from build123d import *

# Parameters (mm, degrees)
SKETCH_1_R             = 10
EXTRUDE_1_DEPTH        = 177
HOLE_WIZARD_M8_1_D     = 6.8
HOLE_WIZARD_M8_1_DEPTH = 19.75
HOLE_WIZARD_M8_1_TIP   = 2.042926105
HOLE_WIZARD_M8_2_D     = 6.8
HOLE_WIZARD_M8_2_DEPTH = 19.75
HOLE_WIZARD_M8_2_TIP   = 2.042926105
CHAMFER_1_SIZE         = 1


with BuildPart() as part:
    # 草图1 → 凸台-拉伸1 (new, symmetric)
    with BuildSketch(Plane.XY):
        Circle(SKETCH_1_R)
    extrude(amount=EXTRUDE_1_DEPTH, both=True)

    # M8 螺纹孔1
    with Locations(Plane(origin=(0, 0, -177), x_dir=(-1, 0, 0), z_dir=(0, 0, -1))):
        with Locations((0, 0)):
            Hole(HOLE_WIZARD_M8_1_D / 2, depth=HOLE_WIZARD_M8_1_DEPTH)
            with Locations((0, 0, -(HOLE_WIZARD_M8_1_DEPTH + HOLE_WIZARD_M8_1_TIP / 2))):  # 118° drill point
                Cone(0, HOLE_WIZARD_M8_1_D / 2, HOLE_WIZARD_M8_1_TIP, mode=Mode.SUBTRACT)

    # M8 螺纹孔2
    with Locations(Plane.XY.offset(177)):
        with Locations((0, 0)):
            Hole(HOLE_WIZARD_M8_2_D / 2, depth=HOLE_WIZARD_M8_2_DEPTH)
            with Locations((0, 0, -(HOLE_WIZARD_M8_2_DEPTH + HOLE_WIZARD_M8_2_TIP / 2))):  # 118° drill point
                Cone(0, HOLE_WIZARD_M8_2_D / 2, HOLE_WIZARD_M8_2_TIP, mode=Mode.SUBTRACT)

    # 倒角1
    chamfer_1_edges = [part.edges().sort_by_distance(p)[0] for p in [
        (-10, 0, -177),
        (-10, 0, 177),
    ]]
    chamfer(chamfer_1_edges, length=CHAMFER_1_SIZE)


solid = part.part
Could you check a few things on this model? Use its own coordinates, in mm. A direction names the side the tool comes from. Coordinates: 2 decimals unless noted, no trailing zeros. Order: outer loops, then holes, each group sorted by start corner. A loop starts at its lowest first (then second) coordinate and runs counter-clockwise, first axis right, second up. Notation, with made-up numbers: (76.25, 18) -> (89.25, 18) arc R26 cw to (89.25, 54) -> close; hole circle Ø9 at (-34, 40.25). An arc over 180 degrees is marked (long way). One line per question, with ' | ' between items.
Q1. On a 3-axis mill with a long thin cutter (end or side, diameter ignored), from which of +Z, -Z, +X, -X, +Y, -Y can I reach the whole of each face in a straight line? I mean faces 1 (the face through (0.74, -3.32, 166.99)), 2 (the face through (0, -4, 177)). Say none if no direction works.
Return value:
face 1: +Z | face 2: +Z, +X, -X, +Y, -Y
Q2. Imagine slicing it at A-A on z = 34.5. Please give me the cut outline in (x, y), and give its area (3 significant figures).
Return value:
outline: circle Ø20 at (0, 0) | area: 314 mm²
Q3. If I drill on L1, parallel to Y at x = 0, z = -164.25; L2, parallel to X at y = 4.5, z = 2.5; L3, parallel to Y at x = 9, z = -55, over which ranges is the centre line in solid material (lowest first)?
Return value:
L1: -10 to -3.4, 3.4 to 10 | L2: -8.93 to 8.93 | L3: -4.36 to 4.36
Q4. Thinking about a two-plate mould opening in X: for faces 3 (the face through (-2.17, -9.76, 2.46)), 4 (the face through (0, -4, -177)), 5 (the face through (-0.74, -3.32, -166.99)), which applies, pulls with the +X half, pulls with the -X half, needs draft (parallel to the pull), parting line crosses it, or undercut?
Return value:
face 3: parting line crosses it | face 4: needs draft | face 5: undercut
Q5. I'm going to push flat-ended pins straight in: P1, Ø6, axis at x = 2, z = 117.5, coming from the -Y side; P2, Ø4, axis at x = 0, y = 0, coming from the -Z side; P3, Ø3, axis at x = -8, z = -114, coming from the -Y side; P4, Ø3, axis at y = 6, z = 43, coming from the +X side. Where does each tip first touch, or does it pass through?
Return value:
P1: y = -10 | P2: z = -156.41 | P3: y = -7.6 | P4: x = 8.93
